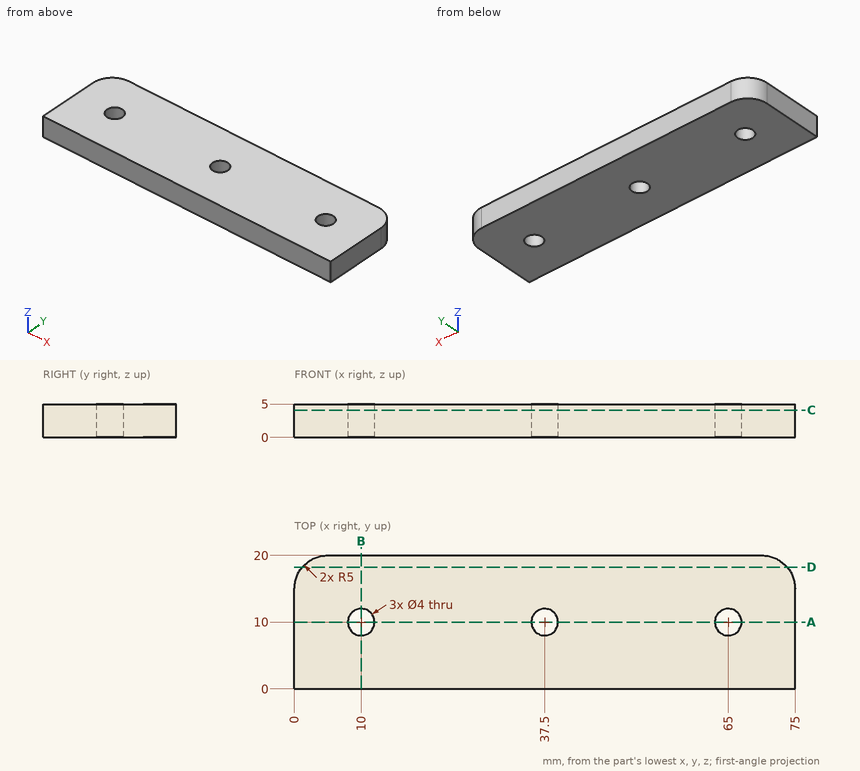
Could you check a few things on this drawing? It's one solid part, dimensions in mm from its lowest x, y, z. Give positions to 0.01 mm unless a question says otherwise; leave off trailing zeros. Loops run counter-clockwise (first coordinate to the right, second up) from the corner with the lowest first, then second, coordinate; pieces in that order, holes last. Notation, with made-up numbers: M 79.5,88.25 L 90.5,88.25 A15 ccw 90.5,108.25 Z; hole C 79,45 d11. An arc over 180 degrees is marked long. Answer as a JSON object with one key per item and string values.
Q1. Suppose I cut it at B-B, the plane x = 10. List the corners of the cut face in (y, z) for me, plus the area to 3 significant figures.
Values found:
{"outline": "M 0,0 L 8,0 L 8,5 L 0,5 Z; M 12,0 L 20,0 L 20,5 L 12,5 Z", "area": "80.0 mm²"}
Q2. Suppose I cut it at A-A, the plane y = 10. List the corners of the cut face in (x, z) for me, plus the area to 3 significant figures.
Values found:
{"outline": "M 0,0 L 8,0 L 8,5 L 0,5 Z; M 12,0 L 35.5,0 L 35.5,5 L 12,5 Z; M 39.5,0 L 63,0 L 63,5 L 39.5,5 Z; M 67,0 L 75,0 L 75,5 L 67,5 Z", "area": "315 mm²"}
Q3. Suppose I cut it at C-C, the plane z = 4.1. List the corners of the cut face in (x, y) for me, plus the area to 3 significant figures.
Values found:
{"outline": "M 0,0 L 75,0 L 75,15 A5 ccw 70,20 L 5,20 A5 ccw 0,15 Z; hole C 10,10 d4; hole C 37.5,10 d4; hole C 65,10 d4", "area": "1,450 mm²"}
Q4. For P1, Ø3, axis at x = 10, y = 10, coming from the -Z side; P2, Ø5, axis at x = 37.5, y = 10, coming from the -Z side, each with a flat end and sliding along its axis, tell me the tip position at first contact or that it passes through.
Values found:
{"P1": "passes through", "P2": "stops at z = 0"}
Q5. Suppose I cut it at D-D, the plane y = 18.25. List the corners of the cut face in (x, z) for me.
Values found:
{"outline": "M 1.2,0 L 73.8,0 L 73.8,5 L 1.2,5 Z"}
Q6. If I drill on probe 1 along Y at (x, z) = (37.5, 1.6); probe 2 along X at (y, z) = (10.5, 0.7); probe 3 along X at (y, z) = (11, 3.3), over which ranges is the centre line in solid material (lowest first)? Write a range as [from, to].
Values found:
{"probe 1": "y = [0, 8], [12, 20]", "probe 2": "x = [0, 8.06], [11.94, 35.56], [39.44, 63.06], [66.94, 75]", "probe 3": "x = [0, 8.27], [11.73, 35.77], [39.23, 63.27], [66.73, 75]"}
